Build history of the part. All positions in model axes, mm. A direction names the side the tool comes from. Coordinates: 2 decimals unless noted, no trailing zeros. Order: outer loops, then holes, each group sorted by start corner. A loop starts at its lowest first (then second) coordinate and runs counter-clockwise, first axis right, second up. Notation, with made-up numbers: M -12,69 L 12,69 A23 ccw 12,105 Z; hole C 14.5,81.25 d4. An arc over 180 degrees is marked long. Use a Markdown table: item, result. Add a question column.
from build123d import *

# Parameters (mm, degrees)
BASE_BLOCK_SKETCH_R              = 10
BASE_BLOCK_SKETCH_R_2            = 7
BASE_BLOCK_DEPTH                 = 14
CLAMP_START                      = -14
CLAMP_RING_DEPTH                 = 14
SIDE_RIB_SKETCH_W                = 3.6
SIDE_RIB_SKETCH_H                = 14
SIDE_RIB_DEPTH                   = 3.5
RIB_START                        = -14
RIB_INFILL_DEPTH                 = 14
MOUNTING_EAR_A_SKETCH_W          = 4
MOUNTING_EAR_A_SKETCH_H          = 13.906308923
MOUNTING_EAR_A_DEPTH             = 3
MOUNTING_EAR_B_SKETCH_W          = 4
MOUNTING_EAR_B_SKETCH_H          = 14
MOUNTING_EAR_B_DEPTH             = 3
CLAMP_SLIT_A_SKETCH_W            = 2
CLAMP_SLIT_A_SKETCH_H            = 2
CLAMP_SLIT_A_DEPTH               = 56
CLAMP_SLIT_B_SKETCH_W            = 2
CLAMP_SLIT_B_SKETCH_H            = 2
CLAMP_SLIT_B_DEPTH               = 92
TRIANGULAR_RELIEF_CUT_DEPTH      = 54
TRIANGULAR_RELIEF_CUT_DEPTH_BACK = 33
TRIANGULAR_RELIEF_SKETCH_R       = 1
RIB_GROOVE_SKETCH_W              = 0.5
RIB_GROOVE_SKETCH_H              = 14
RIB_GROOVE_CUT_DEPTH             = 14
EAR_A_GUSSET_DEPTH               = 1.5
EAR_A_HOLES_SKETCH_R             = 1
EAR_A_HOLES_2X_2_DEPTH           = 6.5
EAR_B_GUSSET_DEPTH               = 1.5
EAR_B_HOLES_SKETCH_R             = 1
EAR_B_HOLES_2X_2_DEPTH           = 10


with BuildPart() as part:
    # Base Block Sketch → Base Block (new body)
    with BuildSketch(Plane(origin=(0, 0, 0), x_dir=(1, 0, 0), z_dir=(0, 1, 0))):
        with Locations(Location((0, 0, 0), (0, 0, 270))):
            Circle(BASE_BLOCK_SKETCH_R)
        with Locations(Location((0, 0, 0), (0, 0, 270))):
            Circle(BASE_BLOCK_SKETCH_R_2, mode=Mode.SUBTRACT)
    extrude(amount=BASE_BLOCK_DEPTH)

    # Clamp Ring Sketch → Clamp Ring (add)
    with BuildSketch(Plane(origin=(0, 14, 0), x_dir=(1, 0, 0), z_dir=(0, 1, 0)).offset(CLAMP_START)):
        with BuildLine():
            Line((-7, -12), (-7, -7.141428429))
            ThreePointArc((-7, -7.141428429), (-9.219544457, -3.872983346), (-10, 0))
            Line((-10, 0), (-10, -12))
            Line((-10, -12), (-7, -12))
        make_face()
        with BuildLine():
            Line((10, -12), (10, 0))
            ThreePointArc((10, 0), (9.219544457, -3.872983346), (7, -7.141428429))
            Line((7, -7.141428429), (7, -12))
            Line((7, -12), (10, -12))
        make_face()
    extrude(amount=CLAMP_RING_DEPTH)



with BuildPart() as body_2:
    # Side Rib Sketch → Side Rib (new, symmetric)
    with BuildSketch(Plane(origin=(0, 0, 0), x_dir=(0, 0, -1), z_dir=(1, 0, 0))):
        with Locations((11.8, 7)):
            Rectangle(SIDE_RIB_SKETCH_W, SIDE_RIB_SKETCH_H)
    extrude(amount=SIDE_RIB_DEPTH, both=True)


with BuildPart() as part_1:
    add(part.part)

    add(body_2.part)  # Rib Infill merges body 2
    # Rib Infill Sketch → Rib Infill (add)
    with BuildSketch(Plane(origin=(0, 14, 0), x_dir=(1, 0, 0), z_dir=(0, 1, 0)).offset(RIB_START)):
        with BuildLine():
            Line((0, 10), (-3.5, 10))
            Line((-3.5, 10), (-3.5, 9.367496998))
            ThreePointArc((-3.5, 9.367496998), (-1.778346145, 9.840603893), (0, 10))
        make_face()
        with BuildLine():
            Line((3.5, 10), (0, 10))
            ThreePointArc((0, 10), (1.778346145, 9.840603893), (3.5, 9.367496998))
            Line((3.5, 9.367496998), (3.5, 10))
        make_face()
    extrude(amount=RIB_INFILL_DEPTH)

    # Mounting Ear A Sketch → Mounting Ear A (add)
    with BuildSketch(Plane.XY.offset(12)):
        with Locations((12, 6.953154462)):
            Rectangle(MOUNTING_EAR_A_SKETCH_W, MOUNTING_EAR_A_SKETCH_H)
    extrude(amount=-MOUNTING_EAR_A_DEPTH)

    # Mounting Ear B Sketch → Mounting Ear B (add)
    with BuildSketch(Plane.XY.offset(12)):
        with Locations((-12, 7)):
            Rectangle(MOUNTING_EAR_B_SKETCH_W, MOUNTING_EAR_B_SKETCH_H)
    extrude(amount=-MOUNTING_EAR_B_DEPTH)

    # Clamp Slit A Sketch → Clamp Slit A (cut)
    with BuildSketch(Plane(origin=(0, 14, 0), x_dir=(1, 0, 0), z_dir=(0, 1, 0))):
        with Locations((-8, -11)):
            Rectangle(CLAMP_SLIT_A_SKETCH_W, CLAMP_SLIT_A_SKETCH_H)
    extrude(amount=-CLAMP_SLIT_A_DEPTH, mode=Mode.SUBTRACT)

    # Clamp Slit B Sketch → Clamp Slit B (cut)
    with BuildSketch(Plane(origin=(0, 14, 0), x_dir=(1, 0, 0), z_dir=(0, 1, 0))):
        with Locations((8, -11)):
            Rectangle(CLAMP_SLIT_B_SKETCH_W, CLAMP_SLIT_B_SKETCH_H)
    extrude(amount=-CLAMP_SLIT_B_DEPTH, mode=Mode.SUBTRACT)

    # Triangular Relief Sketch → Triangular Relief Cut (cut, two sides: drawn at the far end of the back side and taken through both)
    with BuildSketch(Plane(origin=(3.5, 0, 0), x_dir=(0, 0, -1), z_dir=(1, 0, 0)).offset(-TRIANGULAR_RELIEF_CUT_DEPTH_BACK)):
        with Locations((11.483748499, 7)):
            Circle(TRIANGULAR_RELIEF_SKETCH_R)
        with Locations((11.483748499, 3.5)):
            Circle(TRIANGULAR_RELIEF_SKETCH_R)
        with Locations((11.483748499, 10.5)):
            Circle(TRIANGULAR_RELIEF_SKETCH_R)
    extrude(amount=TRIANGULAR_RELIEF_CUT_DEPTH + TRIANGULAR_RELIEF_CUT_DEPTH_BACK, mode=Mode.SUBTRACT)

    # Rib Groove Sketch → Rib Groove Cut (cut)
    with BuildSketch(Plane(origin=(0, 0, -13.6), x_dir=(-1, 0, 0), z_dir=(0, 0, -1))):
        with Locations((0.25, 7)):
            Rectangle(RIB_GROOVE_SKETCH_W, RIB_GROOVE_SKETCH_H)
        with Locations((-0.25, 7)):
            Rectangle(RIB_GROOVE_SKETCH_W, RIB_GROOVE_SKETCH_H)
    extrude(amount=-RIB_GROOVE_CUT_DEPTH, mode=Mode.SUBTRACT)

    # Ear A Gusset Sketch → Ear A Gusset (add, symmetric)
    with BuildSketch(Plane(origin=(0, 7, 0), x_dir=(1, 0, 0), z_dir=(0, 1, 0))):
        Polygon((14, -9), (10, 0), (10, -9), align=None)
    extrude(amount=EAR_A_GUSSET_DEPTH, both=True)

    # Ear A Holes Sketch → Ear A Holes 2xØ2 (cut, symmetric)
    with BuildSketch(Plane(origin=(0, 0, 9), x_dir=(-1, 0, 0), z_dir=(0, 0, -1))):
        with Locations((-12, 11.203154462)):
            Circle(EAR_A_HOLES_SKETCH_R)
        with Locations((-12, 2.75)):
            Circle(EAR_A_HOLES_SKETCH_R)
    extrude(amount=EAR_A_HOLES_2X_2_DEPTH, both=True, mode=Mode.SUBTRACT)

    # Ear B Gusset Sketch → Ear B Gusset (add, symmetric)
    with BuildSketch(Plane(origin=(0, 7, 0), x_dir=(1, 0, 0), z_dir=(0, 1, 0))):
        Polygon((-10, 0), (-14, -9), (-10, -9), align=None)
    extrude(amount=EAR_B_GUSSET_DEPTH, both=True)

    # Ear B Holes Sketch → Ear B Holes 2xØ2 (cut, symmetric)
    with BuildSketch(Plane(origin=(0, 0, 9), x_dir=(-1, 0, 0), z_dir=(0, 0, -1))):
        with Locations((12, 2.5)):
            Circle(EAR_B_HOLES_SKETCH_R)
        with Locations((12, 11.5)):
            Circle(EAR_B_HOLES_SKETCH_R)
    extrude(amount=EAR_B_HOLES_2X_2_DEPTH, both=True, mode=Mode.SUBTRACT)


solid = part_1.part
(1) Drill centre lines: line 1 along Y through (x, z) = (12, 10.05); line 2 along Z through (x, y) = (2.15, 10.5); line 3 along X through (y, z) = (2.5, 0.25). Where is each one in solid material? Low to high. Write a range as from..to.
(2) Slice it at B-B on x = 12. Give the cut face in (y, z).
(3) Slice it at D-D on x = 1.25. Give the cut face in (y, z), and give its area (3 significant figures).
(4) Which spindle directions (+Z, -Z, +X, -X, +Y, -Y) get a long thin tool onto all of the face, cutting with end or side? Do faces 1 (the flat face through (13, 2, 9)), 2 (the flat face through (-9, 7, 11)), 3 (the flat face through (0.5, 7, -10)). Say none if no direction does.
(5) Mould opens along X. For faces 4 (the flat face through (11, 5.5, 6)), 5 (the flat face through (9, 7, 11)), 6 (the flat face through (-10, 11, 4)) say: released by +X, released by -X, zero draft, split by the parting line, or undercut.
(6) Slice it at C-C on z = 0.5. Give the cut face in (x, y).
(7) Slice it at A-A on y = 7. State how many separate pieces and enclosed holes the cut face has, and give its area (3 significant figures).
(8) Drop flat-ended pins along their axis: P1, Ø3, axis at y = 7, z = -11.48, coming from the -X side; P2, Ø2.5, axis at y = 10.5, z = -11.48, coming from the +X side; P3, Ø1.2, axis at y = 3.5, z = -11.48, coming from the +X side; P4, Ø1.2, axis at x = 13, y = 4, coming from the -Z side. Give the stop position or say it passes through.
Solutions:
| question | item | result |
|---|---|---|
| 1 | line 1 | 0..1.75, 3.75..10.2, 12.2..13.91 |
| 1 | line 2 | -13.6..-12.48, -10.48..-6.66, 6.66..9.77 |
| 1 | line 3 | -10..-7, 7..10 |
| 2 | outline | M 0,9 L 1.75,9 L 1.75,12 L 0,12 Z; M 3.75,9 L 5.5,9 L 5.5,4.5 L 8.5,4.5 L 8.5,9 L 10.2,9 L 10.2,12 L 3.75,12 Z; M 12.2,9 L 13.91,9 L 13.91,12 L 12.2,12 Z |
| 3 | outline | M 0,-13.6 L 14,-13.6 L 14,-6.89 L 0,-6.89 Z; M 0,6.89 L 14,6.89 L 14,9.92 L 0,9.92 Z; hole C 3.5,-11.48 d2; hole C 7,-11.48 d2; hole C 10.5,-11.48 d2 |
| 3 | area | 127 mm² |
| 4 | face 1 | -Z, +X, -Y |
| 4 | face 2 | +Z, +Y, -Y |
| 4 | face 3 | -Z, +Y, -Y |
| 5 | face 4 | zero draft |
| 5 | face 5 | undercut |
| 5 | face 6 | released by -X |
| 6 | outline | M -10.22,5.5 L -10,5.5 L -10,0 L -6.98,0 L -6.98,14 L -10,14 L -10,8.5 L -10.22,8.5 Z; M 6.98,0 L 10,0 L 10,5.5 L 10.22,5.5 L 10.22,8.5 L 10,8.5 L 10,14 L 6.98,14 Z |
| 7 | separate pieces | 3 |
| 7 | enclosed holes | 0 |
| 7 | area | 263 mm² |
| 8 | P1 | x = -3.5 |
| 8 | P2 | x = 3.5 |
| 8 | P3 | through |
| 8 | P4 | z = 9 |
